Verification items for the finished model (mm, model axes). Coordinates: 2 decimals unless noted, no trailing zeros. Write each loop counter-clockwise with the first axis right and the second up, starting at its lowest first coordinate (ties: lowest second). Pieces come first, ordered by that corner, then holes.
```python
from build123d import *

# Parameters (mm, degrees)
SKETCH_1_W              = 100
SKETCH_1_H              = 165
EXTRUDE_1_DEPTH         = 10
CHAMFER_1_SIZE          = 2
HOLE_WIZARD_M12_1_D     = 10.2
HOLE_WIZARD_M12_1_DEPTH = 32.75
HOLE_WIZARD_M12_1_TIP   = 3.064389157
HOLE_WIZARD_M8_2_D      = 6.8
HOLE_WIZARD_M8_2_DEPTH  = 22.25
HOLE_WIZARD_M8_2_TIP    = 2.042926105


with BuildPart() as part:
    # 草图1 → 凸台-拉伸1 (new body)
    with BuildSketch(Plane(origin=(0, 0, 0), x_dir=(1, 0, 0), z_dir=(0, 1, 0))):
        with Locations((50, 82.5)):
            Rectangle(SKETCH_1_W, SKETCH_1_H)
    extrude(amount=EXTRUDE_1_DEPTH)

    # 倒角1
    chamfer_1_edges = [part.edges().sort_by_distance(p)[0] for p in [
        (0, 5, -165),
        (100, 5, -165),
        (100, 5, 0),
        (0, 5, 0),
    ]]
    chamfer(chamfer_1_edges, length=CHAMFER_1_SIZE)

    # M12 螺纹孔1
    with Locations(Plane(origin=(35, 10, -135), x_dir=(0, 0, 1), z_dir=(0, 1, 0))):
        with Locations((0, 0)):
            Hole(HOLE_WIZARD_M12_1_D / 2, depth=HOLE_WIZARD_M12_1_DEPTH)
            with Locations((0, 0, -(HOLE_WIZARD_M12_1_DEPTH + HOLE_WIZARD_M12_1_TIP / 2))):  # 118° drill point
                Cone(0, HOLE_WIZARD_M12_1_D / 2, HOLE_WIZARD_M12_1_TIP, mode=Mode.SUBTRACT)

    # M8 螺纹孔2
    with Locations(Plane(origin=(0, 10, 0), x_dir=(1, 0, 0), z_dir=(0, 1, 0))):
        with Locations((13, 60), (13, 15), (87, 15), (87, 60)):
            Hole(HOLE_WIZARD_M8_2_D / 2, depth=HOLE_WIZARD_M8_2_DEPTH)
            with Locations((0, 0, -(HOLE_WIZARD_M8_2_DEPTH + HOLE_WIZARD_M8_2_TIP / 2))):  # 118° drill point
                Cone(0, HOLE_WIZARD_M8_2_D / 2, HOLE_WIZARD_M8_2_TIP, mode=Mode.SUBTRACT)


solid = part.part
```
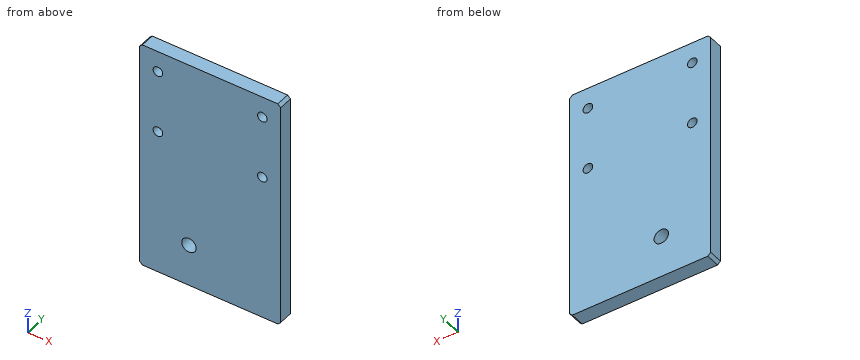
1. Material ranges on L1, parallel to X at y = 4, z = -60; L2, parallel to Z at x = 87, y = 6.75; L3, parallel to X at y = 4.25, z = -135, recorded low to high.
2. Sectioned sample at A-A, the plane x = 13. Record the boundary of the cut face in (y, z).
3. Sectioned sample at C-C, the plane x = 35. Record the boundary of the cut face in (y, z).
4. Gauge pin test, flat end, axial feed: P1, Ø8, axis at x = 35, z = -135, coming from the +Y side. Record the tip position at first contact, or that the pin passes through.
5. Sectioned sample at B-B, the plane z = -135. Record the boundary of the cut face in (x, y), and give its area (3 significant figures).
Outcome:
1. L1: x = 0 to 9.6, 16.4 to 83.6, 90.4 to 100
1. L2: z = -165 to -63.4, -56.6 to -18.4, -11.6 to 0
1. L3: x = 0 to 29.9, 40.1 to 100
2. outline: (0, -165) - (10, -165) - (10, -63.4) - (0, -63.4) - close; (0, -56.6) - (10, -56.6) - (10, -18.4) - (0, -18.4) - close; (0, -11.6) - (10, -11.6) - (10, 0) - (0, 0) - close
3. outline: (0, -165) - (10, -165) - (10, -140.1) - (0, -140.1) - close; (0, -129.9) - (10, -129.9) - (10, 0) - (0, 0) - close
4. P1: passes through
5. outline: (0, 0) - (29.9, 0) - (29.9, 10) - (0, 10) - close; (40.1, 0) - (100, 0) - (100, 10) - (40.1, 10) - close
5. area: 898 mm2
